```python
from build123d import *

# Parameters (mm, degrees)
BOSS_EXTRUDE1_DEPTH = 556
SHELL1_T            = -10
SKETCH2_W           = 100
SKETCH2_H           = 444.236647894
CUT_EXTRUDE1_DEPTH  = 15


with BuildPart() as part:
    # Sketch1 → Boss-Extrude1 (new body)
    with BuildSketch(Plane(origin=(0, 0, 0), x_dir=(1, 0, 0), z_dir=(0, 1, 0))):
        Polygon((100, 0), (500, 0), (500, 60), (-56, 60), (-511.593220339, 241.016949153), (-511.593220339, 121.016949153), (450, -261.044642857), (450, -201.044642857), (100, -61.982142857), align=None)
    extrude(amount=BOSS_EXTRUDE1_DEPTH)

    # Shell1
    shell1_openings = [part.faces().sort_by_distance(p)[0] for p in [
        (450, 278, 231.044642857),
        (-511.593220339, 278, -181.016949153),
        (500, 278, -30),
    ]]
    offset(amount=SHELL1_T, openings=shell1_openings, kind=Kind.INTERSECTION)

    # Sketch2 → Cut-Extrude1 (cut)
    with BuildSketch(Plane(origin=(0, 0, -60), x_dir=(-1, 0, 0), z_dir=(0, 0, -1))):
        with Locations((6, 263.213951143)):
            Rectangle(SKETCH2_W, SKETCH2_H)
    extrude(amount=-CUT_EXTRUDE1_DEPTH, mode=Mode.SUBTRACT)


solid = part.part
```
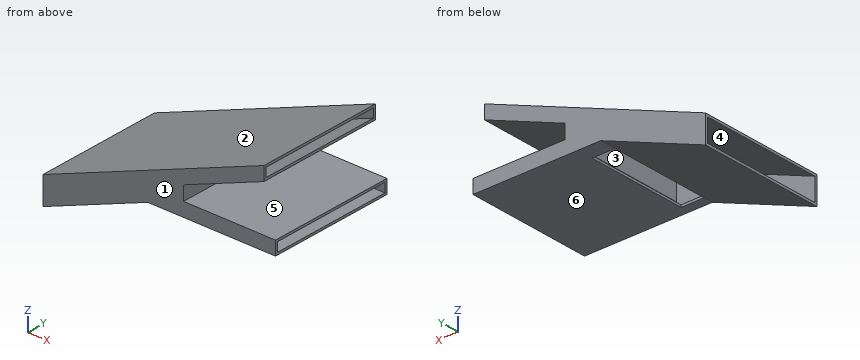
Part model, mm, in its own coordinate system. Face numbers are marked on the shaded views. A direction names the side the tool comes from. Round coordinates to 2 decimals unless told otherwise and drop trailing zeros. Loops run counter-clockwise (first coordinate to the right, second up) from the corner with the lowest first, then second, coordinate; pieces in that order, holes last.
1. Two-plate mould, pull along Z, no slides. Class the marked faces 1, 2 and 3: pulls with the +Z half, pulls with the -Z half, needs draft (parallel to the pull), parting line crosses it, or undercut.
Solutions:
face 1: needs draft
face 2: pulls with the +Z half
face 3: undercut
2. Slice it at A-A (x = 261). Give the cut face in (y, z), and give its area (3 significant figures).
Solutions:
outline: (0, -60) - (556, -60) - (556, 0) - (0, 0) - close; (0, 125.95) - (556, 125.95) - (556, 185.95) - (0, 185.95) - close; hole (10, -50) - (546, -50) - (546, -10) - (10, -10) - close; hole (10, 136.71) - (546, 136.71) - (546, 175.19) - (10, 175.19) - close
area: 24,700 mm2
3. Drill centre lines: line 1 along Z through (x, y) = (332, 172); line 2 along Z through (x, y) = (166.5, 185); line 3 along Y through (x, z) = (-92.5, -52.5). Where is each one in solid material? Low to high.
Solutions:
line 1: z = -60 to -50, -10 to 0, 154.16 to 164.92, 203.4 to 214.16
line 2: z = -60 to -50, -10 to 0, 88.4 to 99.16, 137.64 to 148.4
line 3: y = 0 to 10, 546 to 556
4. Slice it at B-B (y = 171). Give the cut face in (x, z).
Solutions:
outline: (-511.59, -241.02) - (-56, -60) - (-56, -50) - (-57.91, -50) - (-511.59, -230.26) - close; (-511.59, -131.78) - (450, 250.28) - (450, 261.04) - (-511.59, -121.02) - close; (44, -60) - (500, -60) - (500, -50) - (44, -50) - close; (90, -10) - (500, -10) - (500, 0) - (100, 0) - (100, 61.98) - (450, 201.04) - (450, 211.81) - (90, 68.77) - close
5. Slice it at D-D (x = 58.5). Give the cut face in (y, z), and give its area (3 significant figures).
Solutions:
outline: (0, -60) - (556, -60) - (556, 105.49) - (0, 105.49) - close; hole (10, -50) - (546, -50) - (546, 94.73) - (10, 94.73) - close
area: 14,400 mm2
6. Slice it at C-C (z = 32). Give the cut face in (x, y).
Solutions:
outline: (-126.47, 0) - (100, 0) - (100, 556) - (-126.47, 556) - close; hole (-99.39, 10) - (90, 10) - (90, 546) - (-99.39, 546) - close
7. 3-axis set-ups, long thin cutter, end or side, ignore diameter. For the marked faces 4, 5 and 6: which of +Z, -Z, +X, -X, +Y, -Y reach the whole face in a straight line?
Solutions:
face 4: none
face 5: +X, +Y, -Y
face 6: -Z, +X, +Y, -Y
8. Flat gauge pins, fed straight in: pin 1 (8 mm diameter, centred on x = 18, z = -52.5, fed in from -Y); pin 2 (6 mm diameter, centred on x = 70.5, y = 238.5, fed in from -Z); pin 3 (10 mm diameter, centred on x = -257.5, y = 215.5, fed in from +Z); pin 4 (12 mm diameter, centred on x = -115, y = 242.5, fed in from -Z). Where does each tip first touch, or does it go through?
Solutions:
pin 1: stops at y = 0
pin 2: stops at z = -60
pin 3: stops at z = -18.07
pin 4: stops at z = -85.83
